Work out the finished part from the listing and answer in its coordinate system (mm). Face numbers are marked on the shaded views. A direction names the side the tool comes from. Round coordinates to 2 decimals unless told otherwise and drop trailing zeros. Write each loop counter-clockwise with the first axis right and the second up, starting at its lowest first coordinate (ties: lowest second). Pieces come first, ordered by that corner, then holes. Notation, with made-up numbers: M 55,46.5 L 112,46.5 A26 cw 112,78.5 Z; hole C 48.25,37.25 d11. An arc over 180 degrees is marked long. Answer in a Markdown table with one row per item.
```python
from build123d import *

# Parameters (mm, degrees)
LEVER_PROFILE_SKETCH_R         = 32
LEVER_PROFILE_SKETCH_R_2       = 27.5
LEVER_BODY_30MM_DEPTH          = 15
LEVER_PROFILE_SKETCH_R_3       = 19
LEVER_PROFILE_SKETCH_R_4       = 10
LEVER_BODY_30MM_2_DEPTH        = 15
WEB_EXTRUDE_10MM_DEPTH         = 5
BIG_END_HUB_10_15MM_DEPTH      = 10
BIG_END_HUB_10_15MM_DEPTH_BACK = 15
SKETCH1_5_R                    = 27.5
SKETCH1_5_R_2                  = 17
BIG_START                      = 10
SKETCH1_6_R                    = 21.5
SKETCH1_6_R_2                  = 17
BIG_END_SLEEVE_20MM_DEPTH      = 20


with BuildPart() as part:
    # Lever Profile Sketch → Lever Body 30mm (new, symmetric)
    with BuildSketch(Plane.XY):
        Circle(LEVER_PROFILE_SKETCH_R)
        Circle(LEVER_PROFILE_SKETCH_R_2, mode=Mode.SUBTRACT)
    extrude(amount=LEVER_BODY_30MM_DEPTH, both=True)



with BuildPart() as body_2:
    # Lever Profile Sketch → Lever Body 30mm 2 (new, symmetric)
    with BuildSketch(Plane.XY):
        with Locations((0, 75)):
            Circle(LEVER_PROFILE_SKETCH_R_3)
        with Locations((0, 75)):
            Circle(LEVER_PROFILE_SKETCH_R_4, mode=Mode.SUBTRACT)
    extrude(amount=LEVER_BODY_30MM_2_DEPTH, both=True)


with BuildPart() as part_1:
    add(part.part)

    add(body_2.part)  # Web Extrude 10mm merges body 2
    # Sketch1_4 → Web Extrude 10mm (add, symmetric)
    with BuildSketch(Plane.XY):
        with BuildLine():
            Line((0, 32), (0, 56))
            ThreePointArc((0, 56), (-11.518924537, 59.889924636), (-18.321243986, 69.966907631))
            ThreePointArc((-18.321243986, 69.966907631), (-16.836772686, 42.914041255), (-26.678302647, 17.671111111))
            ThreePointArc((-26.678302647, 17.671111111), (-15.141407538, 28.191093944), (0, 32))
        make_face()
        with BuildLine():
            ThreePointArc((18.321243986, 69.966907631), (11.518924537, 59.889924636), (0, 56))
            Line((0, 56), (0, 32))
            ThreePointArc((0, 32), (15.141407538, 28.191093944), (26.678302647, 17.671111111))
            ThreePointArc((26.678302647, 17.671111111), (16.836772686, 42.914041255), (18.321243986, 69.966907631))
        make_face()
    extrude(amount=WEB_EXTRUDE_10MM_DEPTH, both=True)

    # Sketch1_5 → Big End Hub 10_15mm (add, two sides: drawn at the far end of the back side and taken through both)
    with BuildSketch(Plane.XY.offset(-BIG_END_HUB_10_15MM_DEPTH_BACK)):
        Circle(SKETCH1_5_R)
        Circle(SKETCH1_5_R_2, mode=Mode.SUBTRACT)
    extrude(amount=BIG_END_HUB_10_15MM_DEPTH + BIG_END_HUB_10_15MM_DEPTH_BACK)

    # Sketch1_6 → Big End Sleeve 20mm (add)
    with BuildSketch(Plane.XY.offset(BIG_START)):
        Circle(SKETCH1_6_R)
        Circle(SKETCH1_6_R_2, mode=Mode.SUBTRACT)
    extrude(amount=BIG_END_SLEEVE_20MM_DEPTH)


solid = part_1.part
```
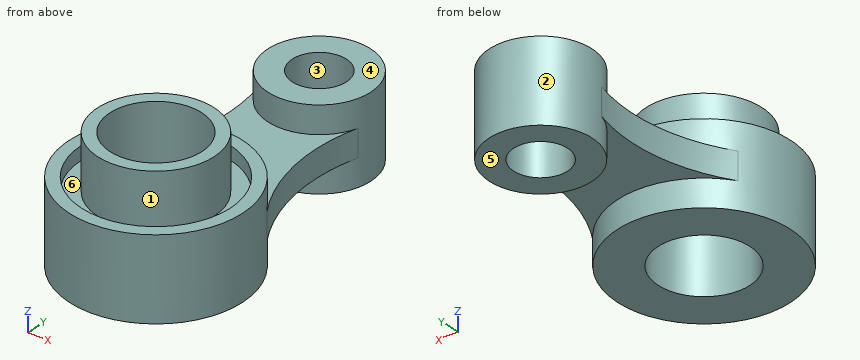
1. The part is cut by section D-D (x = 14.5). Determine the outline of the cut face in (y, z).
Calculated:
| item | result |
|---|---|
| outline | M -28.53,-15 L -8.87,-15 L -8.87,30 L -15.87,30 L -15.87,10 L -23.37,10 L -23.37,15 L -28.53,15 Z; M 8.87,-15 L 28.53,-15 L 28.53,-5 L 62.72,-5 L 62.72,-15 L 87.28,-15 L 87.28,15 L 62.72,15 L 62.72,5 L 28.53,5 L 28.53,15 L 23.37,15 L 23.37,10 L 15.87,10 L 15.87,30 L 8.87,30 Z |
2. The part is cut by section B-B (y = 75). Determine the outline of the cut face in (x, z).
Calculated:
| item | result |
|---|---|
| outline | M -19,-15 L -10,-15 L -10,15 L -19,15 Z; M 10,-15 L 19,-15 L 19,15 L 10,15 Z |
3. The part is cut by section C-C (z = -10). Determine the outline of the cut face in (x, y).
Calculated:
| item | result |
|---|---|
| outline | C 0,0 d64; C 0,75 d38; hole C 0,0 d34; hole C 0,75 d20 |
4. Given pin 1 (16 mm diameter, centred on x = 0, y = 75, fed in from +Z); pin 2 (1 mm diameter, centred on x = -17.5, z = -10, fed in from -Y); pin 3 (3 mm diameter, centred on x = 17.5, z = 22.5, fed in from +Y); pin 4 (10 mm diameter, centred on x = 6.5, z = -9, fed in from -Y), each flat-ended and moving along its own axis, determine where each tip first touches the part or whether it passes through.
Calculated:
| item | result |
|---|---|
| pin 1 | passes through |
| pin 2 | stops at y = -27.11 |
| pin 3 | stops at y = 14.36 |
| pin 4 | stops at y = -31.96 |
5. A tool of negligible diameter and unlimited length cuts with its end or side. For the marked faces 1, 2, 3 and 4, from which of +Z, -Z, +X, -X, +Y, -Y can it reach the whole face along a straight path? Write none if from no direction.
Calculated:
| item | result |
|---|---|
| face 1 | +Z |
| face 2 | none |
| face 3 | +Z, -Z |
| face 4 | +Z, +X, -X, +Y |
6. Consider line 1 along Y through (x, z) = (0, 4.5); line 2 along Y through (x, z) = (0, 6); line 3 along Y through (x, z) = (0, 11). Determine where each line is inside the solid, lowest interval first. Write a range as from..to.
Calculated:
| item | result |
|---|---|
| line 1 | y = -32..-17, 17..65, 85..94 |
| line 2 | y = -32..-17, 17..32, 56..65, 85..94 |
| line 3 | y = -32..-27.5, -21.5..-17, 17..21.5, 27.5..32, 56..65, 85..94 |
7. Determine the mould class of the marked faces 5 and 6 for opening direction Y: released by +Y, released by -Y, zero draft, split by the parting line, or undercut.
Calculated:
| item | result |
|---|---|
| face 5 | zero draft |
| face 6 | undercut |
8. The part is cut by section A-A (x = 0). Determine the outline of the cut face in (y, z).
Calculated:
| item | result |
|---|---|
| outline | M -32,-15 L -17,-15 L -17,30 L -21.5,30 L -21.5,10 L -27.5,10 L -27.5,15 L -32,15 Z; M 17,-15 L 32,-15 L 32,-5 L 56,-5 L 56,-15 L 65,-15 L 65,15 L 56,15 L 56,5 L 32,5 L 32,15 L 27.5,15 L 27.5,10 L 21.5,10 L 21.5,30 L 17,30 Z; M 85,-15 L 94,-15 L 94,15 L 85,15 Z |
